The model under review builds one solid part; all positions refer to its coordinate system, in mm. A direction names the side the tool comes from. Give positions to 0.01 mm unless a question says otherwise; leave off trailing zeros. Write each loop counter-clockwise with the first axis right and the second up, starting at its lowest first coordinate (ties: lowest second). Pieces come first, ordered by that corner, then holes. Notation, with made-up numbers: M 45.25,2.5 L 94.25,2.5 A25 ccw 94.25,20.5 Z; hole C 50,49.5 d7. An arc over 180 degrees is marked long. Write each question's results on one line, items separated by ' | '. Start each with the question number.
from build123d import *

# Parameters (mm, degrees)
SWEEP_THIN1_PROFILE_R   = 15
SWEEP_THIN1_PROFILE_R_2 = 13


with BuildPart() as part:
    # Sweep-Thin1: sweep along a curve in space
    with BuildLine() as sweep_thin1_path:
        Line((-2200, 3201.170909047, 100), (-2200, 3332.935752391, 100))
        ThreePointArc((-2200, 3332.935752391, 100), (-2200, 3361.220023638, 88.284271247), (-2200, 3372.935752391, 60))
        Line((-2200, 3372.935752391, 60), (-2200, 3372.935752391, -6.776695297))
        ThreePointArc((-2200, 3372.935752391, -6.776695297), (-2188.284271248, 3372.935752391, -35.060966545), (-2160, 3372.935752391, -46.776695297))
        Line((-2160, 3372.935752391, -46.776695297), (-397.65799846, 3372.935752391, -46.776695297))
    # Sweep-Thin1 profile (on start of the path) → Sweep-Thin1 (sweep)
    with BuildSketch(Plane(origin=(-2200, 3201.170909047, 100), x_dir=(0, 0, 1), z_dir=(0, 1, 0))):
        Circle(SWEEP_THIN1_PROFILE_R)
        Circle(SWEEP_THIN1_PROFILE_R_2, mode=Mode.SUBTRACT)
    sweep(path=sweep_thin1_path.line)


solid = part.part
(1) Clearance check with flat-ended pins moving along their axes: P1, Ø15.5, axis at x = -2200, y = 3372.94, coming from the +Z side; P2, Ø3, axis at x = -1996, z = -32, coming from the -Y side; P3, Ø15.5, axis at x = -2200, z = 100, coming from the +Y side. State where each tip first meets the part, or that it passes through.
(2) Add section A-A (z = 11.5). State the section outline as (x, y) points, then the cut area to 3 significant figures.
(3) Wall thickness on L1, parallel to Y at x = -2200, z = 17.5; L2, parallel to X at y = 3250, z = 100; L3, parallel to Z at x = -2200, y = 3298.5: over which ranges is each line inside the solid? List them lowest first.
(4) Machinability: for faces 1 (the cylindrical face through (-2214.643, 3369.684, 26.144)), 2 (the flat face through (-397.658, 3366, -58)), 3 (the cylindrical face through (-2214.643, 3267.976, 96.748)), which of the approach directions +Z, -Z, +X, -X, +Y, -Y give a long, thin tool a straight path to every point of the face, cutting with its end or side? Answer none if there is none.
Calculated:
1) P1: stops at z = 104.55 | P2: stops at y = 3365.96 | P3: stops at y = 3377.49
2) outline: C -2200,3372.94 d30; hole C -2200,3372.94 d26 | area: 176 mm²
3) L1: y = 3357.94 to 3359.94, 3385.94 to 3387.94 | L2: x = -2215 to -2213, -2187 to -2185 | L3: z = 85 to 87, 113 to 115
4) face 1: none | face 2: +Z, -Z, +X, +Y, -Y | face 3: -Y
